```python
from build123d import *

# Parameters (mm, degrees)
BASEHEAD_DEPTH = 5.3
SKETCH5_R      = 4
BASEBODY_DEPTH = 35
CHAMFER1_SIZE  = 0.4


with BuildPart() as part:
    # Sketch2 → BaseHead (new body)
    with BuildSketch(Plane(origin=(0, 0, 0), x_dir=(0, 0, -1), z_dir=(1, 0, 0))):
        Polygon((6.5, -3.75277675), (6.5, 3.75277675), (0, 7.505553499), (-6.5, 3.75277675), (-6.5, -3.75277675), (0, -7.505553499), align=None)
    extrude(amount=BASEHEAD_DEPTH)

    # Sketch3 → BearingFace (revolve, cut)
    with BuildSketch(Plane.XY, mode=Mode.PRIVATE) as bearingface_sk:
        Polygon((5.3, 7.505553499), (5.3, 3.44), (4.7, 4.04), (4.7, 7.505553499), align=None)
    revolve(bearingface_sk.sketch.rotate(Axis((-0.957090588, 0, 0), (1, 0, 0)), 90), axis=Axis((-0.957090588, 0, 0), (1, 0, 0)), mode=Mode.SUBTRACT)

    # Sketch4 → HeadChamfer (revolve, cut)
    with BuildSketch(Plane.XY):
        Polygon((0, 7.505553499), (0.365991543, 7.505553499), (0, 6.5), align=None)
    revolve(axis=Axis((-0.493528746, 0, 0), (1, 0, 0)), mode=Mode.SUBTRACT)

    # Sketch5 → BaseBody (add)
    with BuildSketch(Plane(origin=(5.3, 0, 0), x_dir=(0, 0, -1), z_dir=(1, 0, 0))):
        Circle(SKETCH5_R)
    extrude(amount=BASEBODY_DEPTH)

    # Chamfer1
    chamfer1_edges = [part.edges().sort_by_distance(p)[0] for p in [
        (40.3, 0, 4),
    ]]
    chamfer(chamfer1_edges, length=CHAMFER1_SIZE)


solid = part.part
```
Design review of the part built by this model. Coordinates are the model's own, in mm. A direction names the side the tool comes from. Round coordinates to 2 decimals unless told otherwise and drop trailing zeros. Order: outer loops, then holes, each group sorted by start corner. A loop starts at its lowest first (then second) coordinate and runs counter-clockwise, first axis right, second up. Notation, with made-up numbers: M 61,49 L 87,49 A33 cw 87,88 Z; hole C -5,59 d8. An arc over 180 degrees is marked long. Put each result on its own line as item: value.
Q1. Consider section A-A (x = 32). State the section outline as (y, z) points, and give its area (3 significant figures).
Reported:
outline: C 0,0 d8
area: 50.3 mm²
Q2. Machinability: for faces 1 (the face through (4.7, 3, 3)), 2 (the face through (2, 0, 6.5)), which of the approach directions +Z, -Z, +X, -X, +Y, -Y give a long, thin tool a straight path to every point of the face, cutting with its end or side? Answer none if there is none.
Reported:
face 1: +X
face 2: +Z, +X, -X, +Y, -Y
Q3. Insertion check: pin 1 Ø4 at (x, y) = (18, -4.5) entering from -Z; pin 2 Ø1 at (x, y) = (26, 2.5) entering from -Z; pin 3 Ø6 at (x, y) = (17.5, 3) entering from -Z. Each pin has a flat end and moves straight along its axis. Give the tip position at first contact, or say it passes through.
Reported:
pin 1: z = -3.12
pin 2: z = -3.46
pin 3: z = -4
Q4. To check wall thickness, follow line 1 (Z direction, x = 22.5, y = -1.75); line 2 (X direction, y = 4.5, z = 4); line 3 (Y direction, x = 11.5, z = 0.25). State the ranges of each line that lie inside material, in increasing order.
Reported:
line 1: -3.6 to 3.6
line 2: 0 to 4.7
line 3: -3.99 to 3.99
